```python
from build123d import *

# Parameters (mm, degrees)
BASE_PLATE_SKETCH_W    = 80
BASE_PLATE_SKETCH_H    = 115
BASE_PLATE_DEPTH       = 12
BACK_WALL_SKETCH_W     = 80
BACK_WALL_SKETCH_H     = 30
BACK_WALL_DEPTH        = 44
WALL_SLOT_CUT_DEPTH    = 90.678592763
BOSS_PAD_SKETCH_R      = 6
BOSS_PAD_DEPTH         = 20
COUNTERBORE_SKETCH_R   = 17
COUNTERBORE_34X5_DEPTH = 5
BORE_SKETCH_R          = 8
BORE_16_DEPTH          = 15
SUPPORT_RIB_8MM_REACH  = 91.679
RIB_SKETCH_WALL_W      = 218.235363356
RIB_SKETCH_WALL_H      = 8


with BuildPart() as part:
    # Base Plate Sketch → Base Plate (new body)
    with BuildSketch(Plane(origin=(0, 0, 0), x_dir=(1, 0, 0), z_dir=(0, 1, 0))):
        Rectangle(BASE_PLATE_SKETCH_W, BASE_PLATE_SKETCH_H)
    extrude(amount=BASE_PLATE_DEPTH)

    # Back Wall Sketch → Back Wall (add)
    with BuildSketch(Plane(origin=(0, 12, 0), x_dir=(1, 0, 0), z_dir=(0, 1, 0))):
        with Locations((0, 42.5)):
            Rectangle(BACK_WALL_SKETCH_W, BACK_WALL_SKETCH_H)
    extrude(amount=BACK_WALL_DEPTH)

    # Wall Slot Sketch → Wall Slot Cut (cut, through all)
    with BuildSketch(Plane(origin=(0, 56, 0), x_dir=(1, 0, 0), z_dir=(0, 1, 0))):
        Polygon((-24, 57.5), (-24, 47.5), (-32, 47.5), (-32, 37.5), (32, 37.5), (32, 47.5), (24, 47.5), (24, 57.5), align=None)
    extrude(amount=-WALL_SLOT_CUT_DEPTH, mode=Mode.SUBTRACT)

    # Boss Pad Sketch → Boss Pad (add)
    with BuildSketch(Plane(origin=(0, 12, 0), x_dir=(1, 0, 0), z_dir=(0, 1, 0))):
        with BuildLine():
            Line((-40, 27.5), (40, 27.5))
            Line((40, 27.5), (40, -0.5))
            Line((40, -0.5), (24, -0.5))
            Line((24, -0.5), (24, -28))
            ThreePointArc((24, -28), (0, -52), (-24, -28))
            Line((-24, -28), (-24, -0.5))
            Line((-24, -0.5), (-40, -0.5))
            Line((-40, -0.5), (-40, 27.5))
        make_face()
        with Locations(Location((-24, 13.5, 0), (0, 0, 270))):
            Circle(BOSS_PAD_SKETCH_R, mode=Mode.SUBTRACT)
        with Locations(Location((24, 13.5, 0), (0, 0, 270))):
            Circle(BOSS_PAD_SKETCH_R, mode=Mode.SUBTRACT)
    extrude(amount=BOSS_PAD_DEPTH)

    # Counterbore Sketch → Counterbore Ø34x5 (cut)
    with BuildSketch(Plane(origin=(0, 32, 0), x_dir=(1, 0, 0), z_dir=(0, 1, 0))):
        with Locations(Location((0, -28, 0), (0, 0, 270))):
            Circle(COUNTERBORE_SKETCH_R)
    extrude(amount=-COUNTERBORE_34X5_DEPTH, mode=Mode.SUBTRACT)

    # Bore Sketch → Bore Ø16 (cut)
    with BuildSketch(Plane(origin=(0, 27, 0), x_dir=(1, 0, 0), z_dir=(0, 1, 0))):
        with Locations(Location((0, -28, 0), (0, 0, 270))):
            Circle(BORE_SKETCH_R)
    extrude(amount=-BORE_16_DEPTH, mode=Mode.SUBTRACT)

    # Rib Sketch wall → Support Rib 8mm (add, up to next)
    with BuildSketch(Plane(origin=(0, 44, -13.5), x_dir=(0, -0.650791373456, 0.759256602365), z_dir=(0, -0.759256602365, -0.650791373456)), mode=Mode.PRIVATE) as support_rib_8mm_sk1:
        Rectangle(RIB_SKETCH_WALL_W, RIB_SKETCH_WALL_H)
    support_rib_8mm_tool1 = extrude(support_rib_8mm_sk1.sketch, amount=SUPPORT_RIB_8MM_REACH, mode=Mode.PRIVATE) - part.part
    add(support_rib_8mm_tool1.solids().sort_by_distance((0, 44, -13.5))[0])


solid = part.part
```
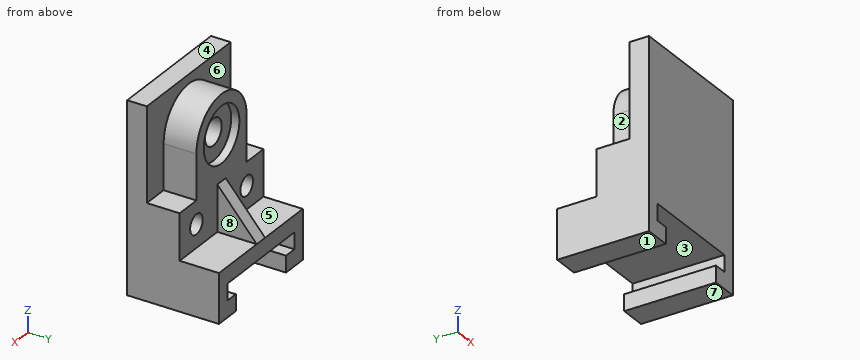
Could you check a few things on this model? Use its own coordinates, in mm. Face numbers are marked on the shaded views. A direction names the side the tool comes from. Give positions to 0.01 mm unless a question says otherwise; leave off trailing zeros. Order: outer loops, then holes, each group sorted by start corner. A loop starts at its lowest first (then second) coordinate and runs counter-clockwise, first axis right, second up.
Q1. Suppose I cut it at C-C, the plane x = 0. Write out the boundary of the cut face in (y, z).
Q2. For the marked faces 5, 6, 7 and 8, which set-ups out of +Z, -Z, +X, -X, +Y, -Y let a thin tool reach every point of the face, with its end or its side?
Q3. Suppose I cut it at D-D, the plane z = 46.5. Write out the boundary of the cut face in (x, y), and give its area (3 significant figures).
Q4. If I drill on line 1 along X through (y, z) = (26.75, -13.5); line 2 along X through (y, z) = (21, 28); line 3 along Z through (x, y) = (27.5, 5), over which ranges is the centre line in solid material (lowest first)?
Q5. Suppose I cut it at A-A, the plane z = -13.5. Write out the boundary of the cut face in (x, y).
Q6. Suppose I cut it at B-B, the plane y = 21. Write out the boundary of the cut face in (x, z), and give its area (3 significant figures).
Q7. I'm going to push flat-ended pins straight in: P1, Ø12, axis at x = -27.5, y = 42, coming from the +Z side; P2, Ø7, axis at y = 49.5, z = -18.5, coming from the -X side; P3, Ø12, axis at y = 45, z = -13.5, coming from the +X side. Where does each tip first touch, or does it pass through?
Q8. We'd pull the mould along Z, two halves only. Please class the marked faces 1, 2, 3 and 4: +Z half, -Z half, draft (parallel to the pull), parting line (faces both ways), or undercut.
Solution:
1. outline: (0, -37.5) - (56, -37.5) - (56, -27.5) - (32, 0.5) - (32, 11) - (27, 11) - (27, 20) - (12, 20) - (12, 36) - (27, 36) - (27, 45) - (32, 45) - (32, 52) - (12, 52) - (12, 57.5) - (0, 57.5) - close
2. face 5: +Z, -X, +Y
2. face 6: +Z, +Y
2. face 7: -Z, +X, -X, +Y, -Y
2. face 8: +Z, +X, +Y
3. outline: (-40, 0) - (40, 0) - (40, 12) - (15.29, 12) - (15.29, 32) - (-15.29, 32) - (-15.29, 12) - (-40, 12) - close
3. area: 1,570 mm2
4. line 1: x = -40 to -30, -18 to 18, 30 to 40
4. line 2: x = -24 to -8, 8 to 24
4. line 3: z = -57.5 to -47.5, -37.5 to 57.5
5. outline: (-40, 0) - (40, 0) - (40, 32) - (30, 32) - (30, 12) - (18, 12) - (18, 32) - (4, 32) - (4, 44) - (-4, 44) - (-4, 32) - (-18, 32) - (-18, 12) - (-30, 12) - (-30, 32) - (-40, 32) - close
6. outline: (-40, -57.5) - (-24, -57.5) - (-24, -47.5) - (-32, -47.5) - (-32, -37.5) - (32, -37.5) - (32, -47.5) - (24, -47.5) - (24, -57.5) - (40, -57.5) - (40, 0.5) - (24, 0.5) - (24, 28) arc R24 ccw to (-24, 28) - (-24, 0.5) - (-40, 0.5) - close; hole circle Ø12 at (-24, -13.5); hole circle Ø16 at (0, 28); hole circle Ø12 at (24, -13.5)
6. area: 5,320 mm2
7. P1: stops at z = -27.5
7. P2: stops at x = -4
7. P3: stops at x = 4
8. face 1: -Z half
8. face 2: draft
8. face 3: undercut
8. face 4: +Z half
